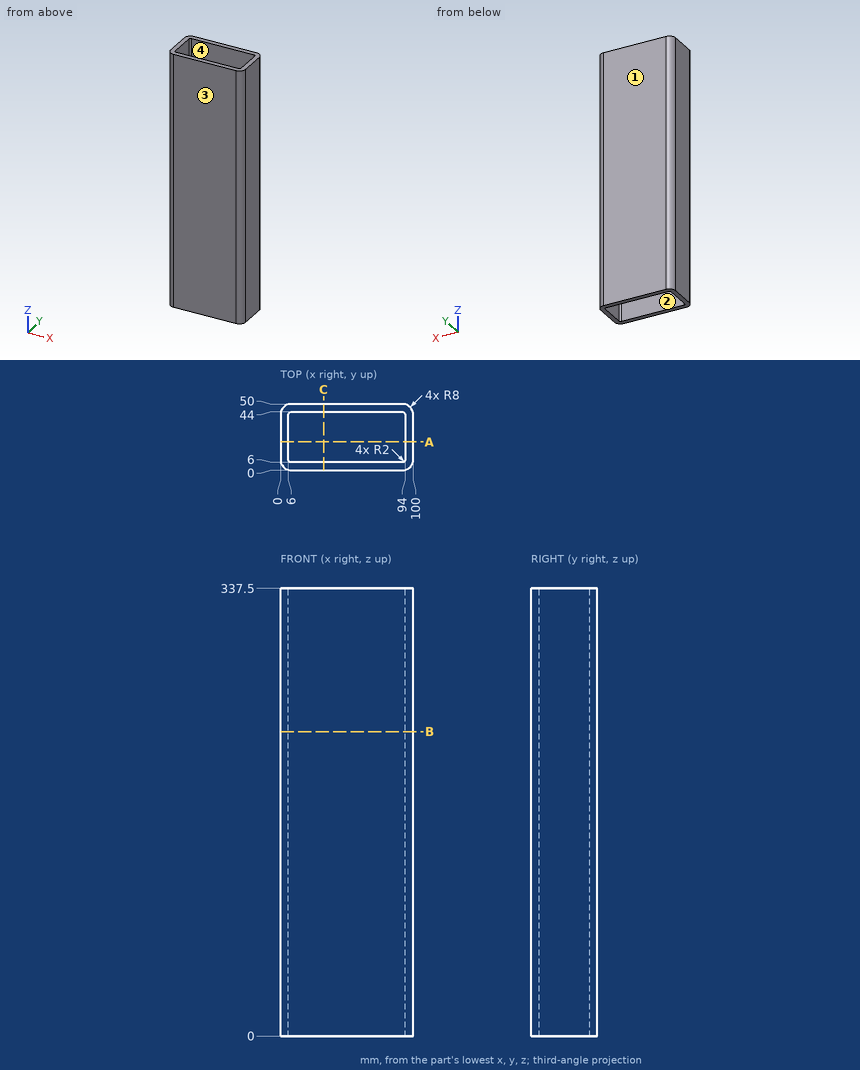
Study the drawing (mm; zero at the part's minimum x, y, z) and answer. Give positions to 0.01 mm unless a question says otherwise; leave off trailing zeros. Write each loop counter-clockwise with the first axis right and the second up, starting at its lowest first coordinate (ties: lowest second). Pieces come first, ordered by that corner, then holes. Notation, with made-up numbers: (-7, -10) - (31, -10) arc R20 ccw to (31, 24) - close; hole circle Ø6 at (78.5, 29.25). An arc over 180 degrees is marked (long way). Use a Markdown table: item, result.
1. For a pull along Y with two mould halves and no side action, classify the marked faces 1, 2, 3 and 4 as released by +Y, released by -Y, zero draft, split by the parting line, or undercut.
Values follow:
| item | result |
|---|---|
| face 1 | released by +Y |
| face 2 | undercut |
| face 3 | released by -Y |
| face 4 | undercut |
2. Section C-C on x = 32.5 is taken. Write down the section's boundary in (y, z).
Values follow:
| item | result |
|---|---|
| outline | (0, 0) - (6, 0) - (6, 337.5) - (0, 337.5) - close; (44, 0) - (50, 0) - (50, 337.5) - (44, 337.5) - close |
3. Find the intervals of material crossed by probe 1 along X at (y, z) = (14, 181); probe 2 along Y at (x, z) = (69, 291); probe 3 along Y at (x, z) = (6.5, 88), in increasing order. Write a range as from..to.
Values follow:
| item | result |
|---|---|
| probe 1 | x = 0..6, 94..100 |
| probe 2 | y = 0..6, 44..50 |
| probe 3 | y = 0.14..6.68, 43.32..49.86 |
4. Section B-B on z = 229.5 is taken. Write down the section's boundary in (x, y), plus the area to 3 significant figures.
Values follow:
| item | result |
|---|---|
| outline | (0, 8) arc R8 ccw to (8, 0) - (92, 0) arc R8 ccw to (100, 8) - (100, 42) arc R8 ccw to (92, 50) - (8, 50) arc R8 ccw to (0, 42) - close; hole (6, 8) arc R2 ccw to (8, 6) - (92, 6) arc R2 ccw to (94, 8) - (94, 42) arc R2 ccw to (92, 44) - (8, 44) arc R2 ccw to (6, 42) - close |
| area | 1,600 mm² |
5. Section A-A on y = 21.5 is taken. Write down the section's boundary in (x, z), plus the area to 3 significant figures.
Values follow:
| item | result |
|---|---|
| outline | (0, 0) - (6, 0) - (6, 337.5) - (0, 337.5) - close; (94, 0) - (100, 0) - (100, 337.5) - (94, 337.5) - close |
| area | 4,050 mm² |
